```python
from build123d import *

# Parameters (mm, degrees)
SKETCH1_W                   = 60
SKETCH1_H                   = 40
BOSS_EXTRUDE1_DEPTH         = 37
CHAMFER1_SIZE               = 3
M6_TAPPED_HOLE1_D           = 5
M6_TAPPED_HOLE1_DEPTH       = 12
M6_TAPPED_HOLE1_TIP         = 1.502151548
HOLE1_D                     = 8
HOLE1_DEPTH                 = 10
HOLE2_D                     = 8
HOLE2_DEPTH                 = 10
M6_TAPPED_HOLE2_D           = 5
M6_TAPPED_HOLE2_DEPTH       = 12
M6_TAPPED_HOLE2_CSINK_D     = 6.05
M6_TAPPED_HOLE2_CSINK_ANGLE = 90
M6_TAPPED_HOLE2_TIP         = 1.502151548


with BuildPart() as part:
    # Sketch1 → Boss-Extrude1 (new body)
    with BuildSketch(Plane.XY):
        with Locations((-4.502067899, 30.192307692)):
            Rectangle(SKETCH1_W, SKETCH1_H)
    extrude(amount=BOSS_EXTRUDE1_DEPTH)

    # Chamfer1
    chamfer1_edges = [part.edges().sort_by_distance(p)[0] for p in [
        (-34.502067899, 50.192307692, 18.5),
        (25.497932101, 50.192307692, 18.5),
        (25.497932101, 10.192307692, 18.5),
        (-34.502067899, 10.192307692, 18.5),
    ]]
    chamfer(chamfer1_edges, length=CHAMFER1_SIZE)

    # M6 Tapped Hole1
    with Locations(Plane.XY.offset(37)):
        with Locations((-24.502067899, 42.192307692), (15.497932101, 18.192307692)):
            Hole(M6_TAPPED_HOLE1_D / 2, depth=M6_TAPPED_HOLE1_DEPTH)
            with Locations((0, 0, -(M6_TAPPED_HOLE1_DEPTH + M6_TAPPED_HOLE1_TIP / 2))):  # 118° drill point
                Cone(0, M6_TAPPED_HOLE1_D / 2, M6_TAPPED_HOLE1_TIP, mode=Mode.SUBTRACT)

    # Hole1
    with Locations(Plane.XY.offset(37)):
        with Locations((15.497932101, 42.192307692), (-24.502067899, 18.192307692)):
            Hole(HOLE1_D / 2, depth=HOLE1_DEPTH)

    # Hole2
    with Locations(Plane(origin=(0, 0, 0), x_dir=(-1, 0, 0), z_dir=(0, 0, -1))):
        with Locations((24.502067899, 42.192307692), (-15.497932101, 18.192307692)):
            Hole(HOLE2_D / 2, depth=HOLE2_DEPTH)

    # M6 Tapped Hole2
    with Locations(Plane(origin=(0, 0, 0), x_dir=(-1, 0, 0), z_dir=(0, 0, -1))):
        with Locations((-15.497932101, 42.192307692), (24.502067899, 18.192307692)):
            CounterSinkHole(M6_TAPPED_HOLE2_D / 2, M6_TAPPED_HOLE2_CSINK_D / 2, depth=M6_TAPPED_HOLE2_DEPTH, counter_sink_angle=M6_TAPPED_HOLE2_CSINK_ANGLE)
            with Locations((0, 0, -(M6_TAPPED_HOLE2_DEPTH + M6_TAPPED_HOLE2_TIP / 2))):  # 118° drill point
                Cone(0, M6_TAPPED_HOLE2_D / 2, M6_TAPPED_HOLE2_TIP, mode=Mode.SUBTRACT)


solid = part.part
```
Geometry: final body of the model. Coordinates: model frame, mm. A direction names the side the tool comes from. Coordinates: 2 decimals unless noted, no trailing zeros. Loops run counter-clockwise (first coordinate to the right, second up) from the corner with the lowest first, then second, coordinate; pieces in that order, holes last. Notation, with made-up numbers: M -20.75,-31.75 L -8.75,-31.75 A36 cw -8.75,5.25 Z; hole C 6.5,17.25 d10. An arc over 180 degrees is marked long. Put each result on its own line as item: value.
(1) Material intervals for probe 1 along Y at (x, z) = (16, 32.5); probe 2 along X at (y, z) = (17.5, 12); probe 3 along X at (y, z) = (14.5, 33), sorted ascending.
Answer sheet:
probe 1: y = 10.19 to 15.74, 20.64 to 38.22, 46.16 to 50.19
probe 2: x = -34.5 to -26.9, -22.1 to 25.5
probe 3: x = -34.5 to -26.04, -22.96 to 25.5
(2) Cut plane B-B on z = 32. Return the cut outline in (x, y).
Answer sheet:
outline: M -34.5,13.19 L -31.5,10.19 L 22.5,10.19 L 25.5,13.19 L 25.5,47.19 L 22.5,50.19 L -31.5,50.19 L -34.5,47.19 Z; hole C -24.5,18.19 d8; hole C -24.5,42.19 d5; hole C 15.5,42.19 d8; hole C 15.5,18.19 d5
(3) Draft query along Y for faces 4 (the face through (-34.502, 30, 18)), 5 (the face through (14.98, 22.16, 5.07)), 6 (the face through (-5, 50.192, 18)). Return one class per face: pulls with the +Y half, pulls with the -Y half, needs draft (parallel to the pull), parting line crosses it, or undercut.
Answer sheet:
face 4: needs draft
face 5: undercut
face 6: pulls with the +Y half
(4) Cut plane A-A on z = 26. Return the cut outline in (x, y), then the cut area to 3 significant figures.
Answer sheet:
outline: M -34.5,13.19 L -31.5,10.19 L 22.5,10.19 L 25.5,13.19 L 25.5,47.19 L 22.5,50.19 L -31.5,50.19 L -34.5,47.19 Z; hole C -24.5,42.19 d5; hole C 15.5,18.19 d5
area: 2,340 mm^2
(5) First-contact query: pin 1 (4.5 mm diameter, centred on x = 15.5, y = 18.19, fed in from -Z). Flat tip, straight axial feed; report the tip coordinate or a pass-through.
Answer sheet:
pin 1: stops at z = 10
(6) Access query for faces 1 (the face through (-22.66, 43.88, 30.92)), 2 (the face through (25.498, 30, 18)), 3 (the face through (-24.83, 20.67, 6.34)). Directions: +Z, -Z, +X, -X, +Y, -Y. A direction counts if a zero-diameter tool reaches every point of the face in a straight line with its end or side. Return the directions, or none.
Answer sheet:
face 1: +Z
face 2: +Z, -Z, +X, +Y, -Y
face 3: -Z
